The figure shows three views and two pictorial views of one solid part (mm, origin at its lowest corner). Answer the questions. A direction names the side the tool comes from. Give positions to 0.01 mm unless a question says otherwise; leave off trailing zeros. Order: outer loops, then holes, each group sorted by start corner. A loop starts at its lowest first (then second) coordinate and runs counter-clockwise, first axis right, second up. Notation, with made-up numbers: M 37.25,75 L 91.25,75 A20 cw 91.25,114 Z; hole C 82.25,64 d6. An arc over 180 degrees is marked long. One line per item, written item: value.
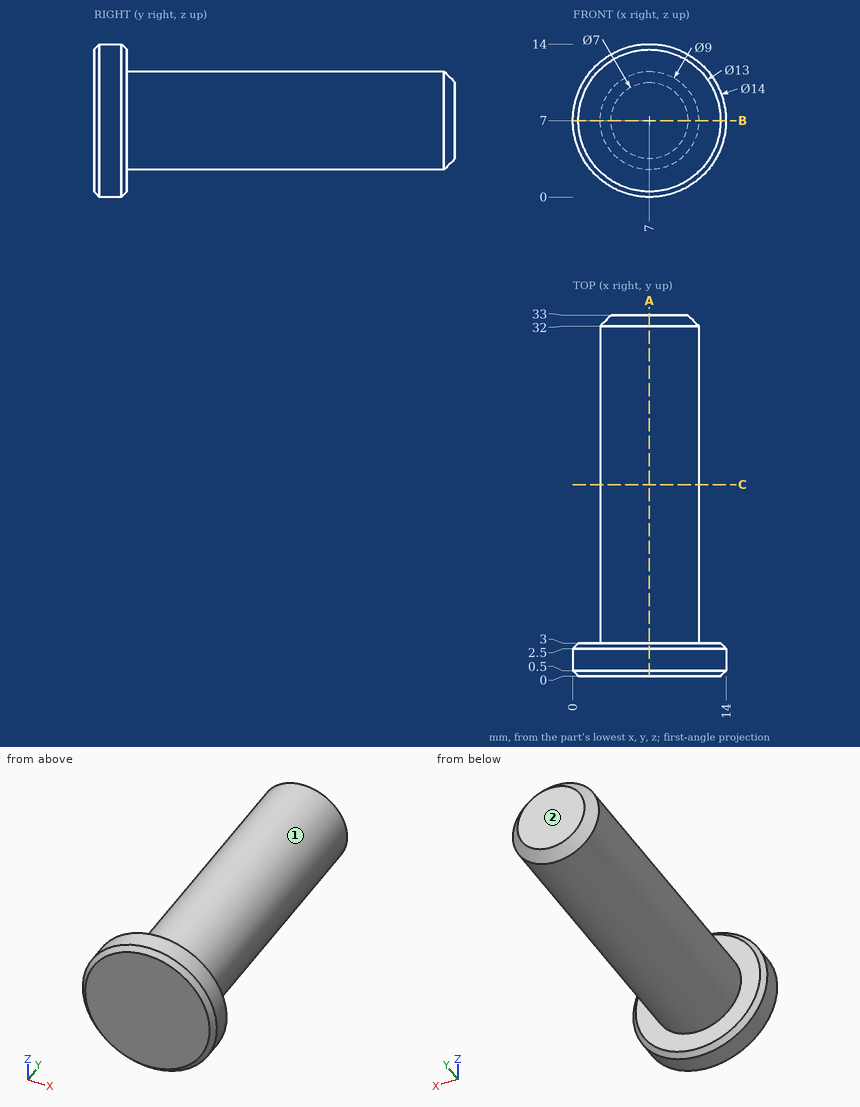
1) Find section B-B, the plane z = 7. Write down the section's boundary in (x, y).
Reported:
outline: M 0,0.5 L 0.5,0 L 13.5,0 L 14,0.5 L 14,2.5 L 13.5,3 L 11.5,3 L 11.5,32 L 10.5,33 L 3.5,33 L 2.5,32 L 2.5,3 L 0.5,3 L 0,2.5 Z
2) Each of these flat-tipped pins is pushed along its axis until it touches: pin 1 Ø4 at (y, z) = (9, 12.5) entering from -X; pin 2 Ø4 at (x, y) = (3.5, 11.5) entering from -Z; pin 3 Ø1 at (x, z) = (12, 1.5) entering from -Y; pin 4 Ø6 at (x, z) = (10, 3) entering from +Y. Where does it stop, or does it pass through?
Reported:
pin 1: stops at x = 4.17
pin 2: stops at z = 2.76
pin 3: stops at y = 0.43
pin 4: stops at y = 33
3) Which of the six approach directions +Z, -Z, +X, -X, +Y, -Y give full straight-line access (tool end or side, diameter ignored) to the marked faces 1 and 2?
Reported:
face 1: +Y
face 2: +Z, -Z, +X, -X, +Y
4) Consider probe 1 along Y at (x, z) = (6.25, 1); probe 2 along Z at (x, y) = (7.25, 20); probe 3 along X at (y, z) = (8, 5.75). Determine where each line is inside the solid, lowest interval first.
Reported:
probe 1: y = 0 to 3
probe 2: z = 2.51 to 11.49
probe 3: x = 2.68 to 11.32
5) Find section A-A, the plane x = 7. Write down the section's boundary in (y, z).
Reported:
outline: M 0,0.5 L 0.5,0 L 2.5,0 L 3,0.5 L 3,2.5 L 32,2.5 L 33,3.5 L 33,10.5 L 32,11.5 L 3,11.5 L 3,13.5 L 2.5,14 L 0.5,14 L 0,13.5 Z
6) Find section C-C, the plane y = 17.5. Write down the section's boundary in (x, z).
Reported:
outline: C 7,7 d9
